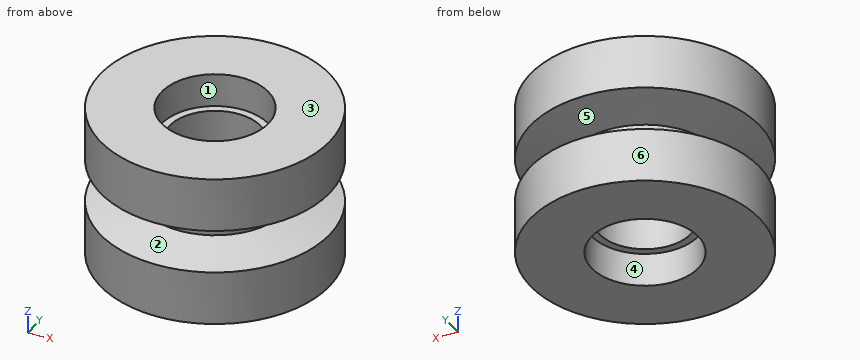
from build123d import *

# Parameters (mm, degrees)
SKETCH_1_R          = 37.5
SKETCH_1_R_2        = 15
EXTRUDE_1_DEPTH     = 50
SKETCH_3_R          = 17.5
CUT_EXTRUDE_1_DEPTH = 11
CUT_EXTRUDE_START   = -11
SKETCH_4_R          = 17.5
CUT_EXTRUDE_2_DEPTH = 11


with BuildPart() as part:
    # 草图1 → 凸台-拉伸1 (new body)
    with BuildSketch(Plane.XY):
        Circle(SKETCH_1_R)
        Circle(SKETCH_1_R_2, mode=Mode.SUBTRACT)
    extrude(amount=EXTRUDE_1_DEPTH)

    # 草图2 → 切除-旋转1 (revolve, cut)
    with BuildSketch(Plane(origin=(0, 0, 0), x_dir=(1, 0, 0), z_dir=(0, 1, 0))):
        Polygon((-38.25, -17.648818614), (-23.25, -21.25), (-23.25, -28.75), (-38.25, -32.351181386), align=None)
    revolve(axis=Axis((0, 0, 0), (0, 0, 1)), mode=Mode.SUBTRACT)

    # 草图3 → 切除-拉伸1 (cut)
    with BuildSketch(Plane.XY.offset(50)):
        Circle(SKETCH_3_R)
    extrude(amount=-CUT_EXTRUDE_1_DEPTH, mode=Mode.SUBTRACT)

    # 草图4 → 切除-拉伸2 (cut)
    with BuildSketch(Plane(origin=(0, 0, 0), x_dir=(-1, 0, 0), z_dir=(0, 0, -1)).offset(CUT_EXTRUDE_START)):
        with Locations(Location((0, 0, 0), (0, 0, 180))):
            Circle(SKETCH_4_R)
    extrude(amount=CUT_EXTRUDE_2_DEPTH, mode=Mode.SUBTRACT)


solid = part.part
Here's how the part is built. I have some questions about the finished solid (model axes, mm). Face numbers are marked on the shaded views. A direction names the side the tool comes from. Coordinates: 2 decimals unless noted, no trailing zeros. Order: outer loops, then holes, each group sorted by start corner. A loop starts at its lowest first (then second) coordinate and runs counter-clockwise, first axis right, second up. Notation, with made-up numbers: (25, 35.5) -> (65, 35.5) arc R27 cw to (65, 70.5) -> close; hole circle Ø4 at (-31, 64). An arc over 180 degrees is marked (long way). Answer in a Markdown table with one row per item.
(1) I want a section at A-A on y = 0. List the corners of the cut face in (x, z) for me.
Answer key:
| item | result |
|---|---|
| outline | (-37.5, 0) -> (-17.5, 0) -> (-17.5, 11) -> (-15, 11) -> (-15, 39) -> (-17.5, 39) -> (-17.5, 50) -> (-37.5, 50) -> (-37.5, 32.17) -> (-23.25, 28.75) -> (-23.25, 21.25) -> (-37.5, 17.83) -> close; (15, 11) -> (17.5, 11) -> (17.5, 0) -> (37.5, 0) -> (37.5, 17.83) -> (23.25, 21.25) -> (23.25, 28.75) -> (37.5, 32.17) -> (37.5, 50) -> (17.5, 50) -> (17.5, 39) -> (15, 39) -> close |
(2) I want a section at C-C on z = 34. List the corners of the cut face in (x, y) for me, then the cut area to 3 significant figures.
Answer key:
| item | result |
|---|---|
| outline | circle Ø75 at (0, 0); hole circle Ø30 at (0, 0) |
| area | 3,710 mm^2 |
(3) On a 3-axis mill with a long thin cutter (end or side, diameter ignored), from which of +Z, -Z, +X, -X, +Y, -Y can I reach the whole of each face in a straight line? I mean the marked faces 4, 5 and 6. Say none if no direction works.
Answer key:
| item | result |
|---|---|
| face 4 | -Z |
| face 5 | none |
| face 6 | +Z, -Z |
(4) I want a section at D-D on z = 10. List the corners of the cut face in (x, y) for me.
Answer key:
| item | result |
|---|---|
| outline | circle Ø75 at (0, 0); hole circle Ø35 at (0, 0) |
(5) Please list where these lines run through material, in increasing order: probe 1 along Y at (x, z) = (0, 41.75); probe 2 along X at (y, z) = (0, 17); probe 3 along Z at (x, y) = (-15.5, -2).
Answer key:
| item | result |
|---|---|
| probe 1 | -37.5 to -17.5, 17.5 to 37.5 |
| probe 2 | -37.5 to -15, 15 to 37.5 |
| probe 3 | 11 to 39 |
(6) Will these pins go through, and if not, where does the flat tip stop? pin 1 Ø1 at (y, z) = (23.5, 39) entering from -X; pin 2 Ø2 at (y, z) = (-9, 7.5) entering from +X; pin 3 Ø8 at (x, z) = (-24.5, 44) entering from +Y.
Answer key:
| item | result |
|---|---|
| pin 1 | x = -29.62 |
| pin 2 | x = 36.64 |
| pin 3 | y = 31.4 |
(7) Thinking about a two-plate mould opening in Y: for the marked faces 1, 2 and 3, which applies, +Y half, -Y half, draft (parallel to the pull), parting line (faces both ways), or undercut?
Answer key:
| item | result |
|---|---|
| face 1 | undercut |
| face 2 | parting line |
| face 3 | draft |
